Work out the finished part from the listing and answer in its coordinate system (mm). Face numbers are marked on the shaded views. A direction names the side the tool comes from. Give positions to 0.01 mm unless a question says otherwise; leave off trailing zeros. Write each loop counter-clockwise with the first axis right and the second up, starting at its lowest first coordinate (ties: lowest second). Pieces come first, ordered by that corner, then holes. Notation, with made-up numbers: (39.25, -24) -> (90.25, -24) arc R23 ccw to (90.25, -10) -> close; hole circle Ø7 at (70, 23). An arc over 180 degrees is marked (long way). Use a Markdown table: item, result. Add a question column.
Q1. Each of these flat-tipped pins is pushed along its axis until it touches: pin 1 Ø3 at (y, z) = (-24.5, 6.5) entering from +X; pin 2 Ø1 at (y, z) = (-8, 4.5) entering from +X; pin 3 Ø7 at (x, y) = (0, -27.5) entering from +Z. Where does it stop, or does it pass through?
Q2. For a pull along Y with two mould halves and no side action, classify the marked faces 3, 4, 5 and 6 as pulls with the +Y half, pulls with the -Y half, needs draft (parallel to the pull), parting line crosses it, or undercut.
Q3. For the marked faces 1 and 2, determine the directions among +Z, -Z, +X, -X, +Y, -Y from which every point of the face is accessible in a straight line to the end or side of a thin tool.
Q4. Consider line 1 (X direction, y = -29, z = 3); line 2 (Y direction, x = 27, z = 2); line 3 (Y direction, x = 6.5, z = 2.5). Determine where each line is inside the solid, lowest interval first.
Q5. Section C-C, the plane y = -27.5 is taken. Give the vertices of the cut face in (x, z).
Q6. Section A-A, the plane x = 0 is taken. Give the vertices of the cut face in (y, z).
Q7. Section B-B, the plane z = 6.25 is taken. Give the vertices of the cut face in (x, y).
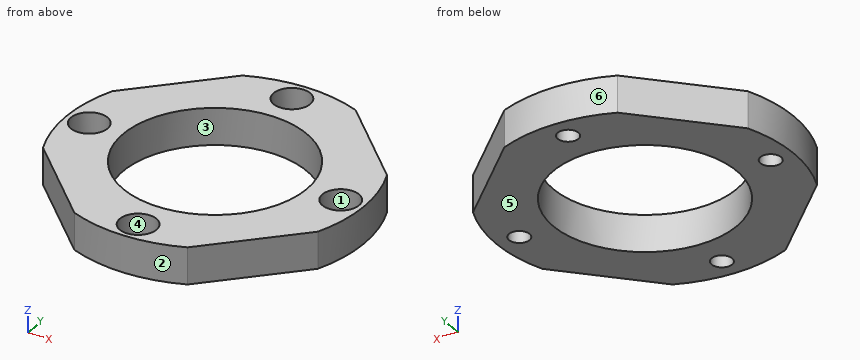
from build123d import *

# Parameters (mm, degrees)
SKETCH1_R                                            = 20
BOSS_EXTRUDE1_DEPTH                                  = 8
HOLE_SIZE_PER_SOCKET_HEAD_CAP_SCREW_TYPE_D           = 4.5
HOLE_SIZE_PER_SOCKET_HEAD_CAP_SCREW_TYPE_CBORE_D     = 8
HOLE_SIZE_PER_SOCKET_HEAD_CAP_SCREW_TYPE_CBORE_DEPTH = 4.6


with BuildPart() as part:
    # Sketch1 → Boss-Extrude1 (new body)
    with BuildSketch(Plane.XY):
        with BuildLine():
            Line((-30.0520382, -12.374368671), (-12.374368671, -30.0520382))
            ThreePointArc((-12.374368671, -30.0520382), (0, -32.5), (12.374368671, -30.0520382))
            Line((12.374368671, -30.0520382), (30.0520382, -12.374368671))
            ThreePointArc((30.0520382, -12.374368671), (32.5, 0), (30.0520382, 12.374368671))
            Line((30.0520382, 12.374368671), (12.374368671, 30.0520382))
            ThreePointArc((12.374368671, 30.0520382), (0, 32.5), (-12.374368671, 30.0520382))
            Line((-12.374368671, 30.0520382), (-30.0520382, 12.374368671))
            ThreePointArc((-30.0520382, 12.374368671), (-32.5, 0), (-30.0520382, -12.374368671))
        make_face()
        Circle(SKETCH1_R, mode=Mode.SUBTRACT)
    extrude(amount=BOSS_EXTRUDE1_DEPTH)

    # Hole size per socket head cap screw type 1 (through all)
    with Locations(Plane.XY.offset(8)):
        with Locations((0, 27.5), (-27.5, 0), (0, -27.5), (27.5, 0)):
            CounterBoreHole(HOLE_SIZE_PER_SOCKET_HEAD_CAP_SCREW_TYPE_D / 2, HOLE_SIZE_PER_SOCKET_HEAD_CAP_SCREW_TYPE_CBORE_D / 2, HOLE_SIZE_PER_SOCKET_HEAD_CAP_SCREW_TYPE_CBORE_DEPTH)


solid = part.part
Result set:
| question | item | result |
|---|---|---|
| 1 | pin 1 | stops at x = 19.43 |
| 1 | pin 2 | stops at x = 31.62 |
| 1 | pin 3 | stops at z = 3.4 |
| 2 | face 3 | undercut |
| 2 | face 4 | undercut |
| 2 | face 5 | needs draft |
| 2 | face 6 | pulls with the +Y half |
| 3 | face 1 | +Z |
| 3 | face 2 | +Z, -Z, -Y |
| 4 | line 1 | x = -13.43 to -1.68, 1.68 to 13.43 |
| 4 | line 2 | y = -15.43 to -2.19, 2.19 to 15.43 |
| 4 | line 3 | y = -31.84 to -18.91, 18.91 to 31.84 |
| 5 | outline | (-14.93, 0) -> (-2.25, 0) -> (-2.25, 3.4) -> (-4, 3.4) -> (-4, 8) -> (-14.93, 8) -> close; (2.25, 0) -> (14.93, 0) -> (14.93, 8) -> (4, 8) -> (4, 3.4) -> (2.25, 3.4) -> close |
| 6 | outline | (-32.5, 0) -> (-29.75, 0) -> (-29.75, 3.4) -> (-31.5, 3.4) -> (-31.5, 8) -> (-32.5, 8) -> close; (-25.25, 0) -> (-20, 0) -> (-20, 8) -> (-23.5, 8) -> (-23.5, 3.4) -> (-25.25, 3.4) -> close; (20, 0) -> (25.25, 0) -> (25.25, 3.4) -> (23.5, 3.4) -> (23.5, 8) -> (20, 8) -> close; (29.75, 0) -> (32.5, 0) -> (32.5, 8) -> (31.5, 8) -> (31.5, 3.4) -> (29.75, 3.4) -> close |
| 7 | outline | (-30.05, -12.37) -> (-12.37, -30.05) arc R32.5 ccw to (12.37, -30.05) -> (30.05, -12.37) arc R32.5 ccw to (30.05, 12.37) -> (12.37, 30.05) arc R32.5 ccw to (-12.37, 30.05) -> (-30.05, 12.37) arc R32.5 ccw to start; hole circle Ø8 at (-27.5, 0); hole circle Ø40 at (0, 0); hole circle Ø8 at (0, -27.5); hole circle Ø8 at (0, 27.5); hole circle Ø8 at (27.5, 0) |
